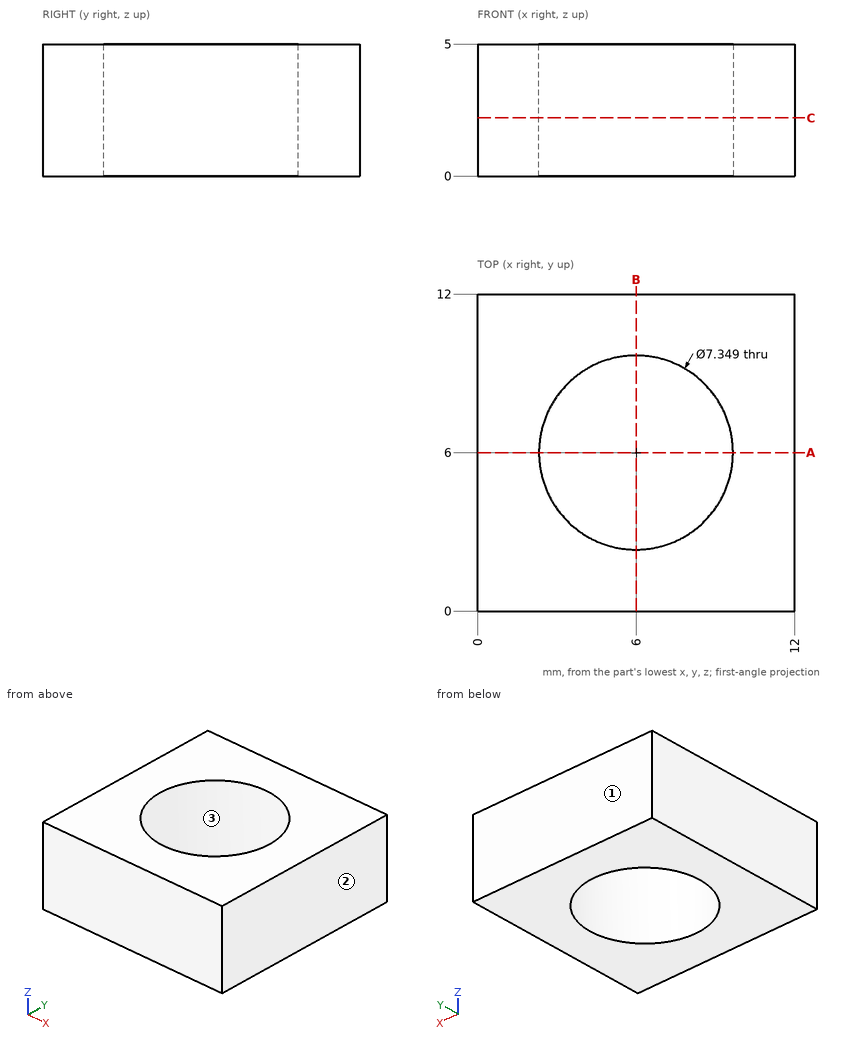
Geometry check sheet. Reference: drawing and pictorial views, mm from the part's lowest x, y, z. Coordinates: 2 decimals unless noted, no trailing zeros. Loops run counter-clockwise (first coordinate to the right, second up) from the corner with the lowest first, then second, coordinate; pieces in that order, holes last. Notation, with made-up numbers: (5, -28) - (50, -28) arc R24 cw to (50, -7) - close; hole circle Ø2 at (-38.5, -39.5). An arc over 180 degrees is marked (long way). Return JSON: item names as keys, results as strings.
1. Section check C-C, the plane z = 2.2. Record the boundary of the cut face in (x, y), then the cut area to 3 significant figures.
Established:
{"outline": "(0, 0) - (12, 0) - (12, 12) - (0, 12) - close; hole circle Ø7.35 at (6, 6)", "area": "102 mm2"}
2. Thickness scan on L1, parallel to Y at x = 6, z = 1.65; L2, parallel to Y at x = 9.25, z = 0.7 (1 decimal); L3, parallel to X at y = 8.5, z = 1.75. Record the ranges inside material, lowest first.
Established:
{"L1": "y = 0 to 2.33, 9.67 to 12", "L2": "y = 0 to 4.3, 7.7 to 12", "L3": "x = 0 to 3.31, 8.69 to 12"}
3. Mould release check, pull along Y, two halves, no side actions. Record for the marked faces 1, 2 and 3: +Y half, -Y half, draft (parallel to the pull), parting line (faces both ways), or undercut.
Established:
{"face 1": "+Y half", "face 2": "draft", "face 3": "undercut"}
4. Section check A-A, the plane y = 6. Record the boundary of the cut face in (x, z).
Established:
{"outline": "(0, 0) - (2.33, 0) - (2.33, 5) - (0, 5) - close; (9.67, 0) - (12, 0) - (12, 5) - (9.67, 5) - close"}
5. Go/stop test with a flat-tipped pin: pin 1 (6 mm diameter, centred on x = 7, y = 8, fed in from -Z). Record where the tip stops, or that it passes through.
Established:
{"pin 1": "stops at z = 0"}
